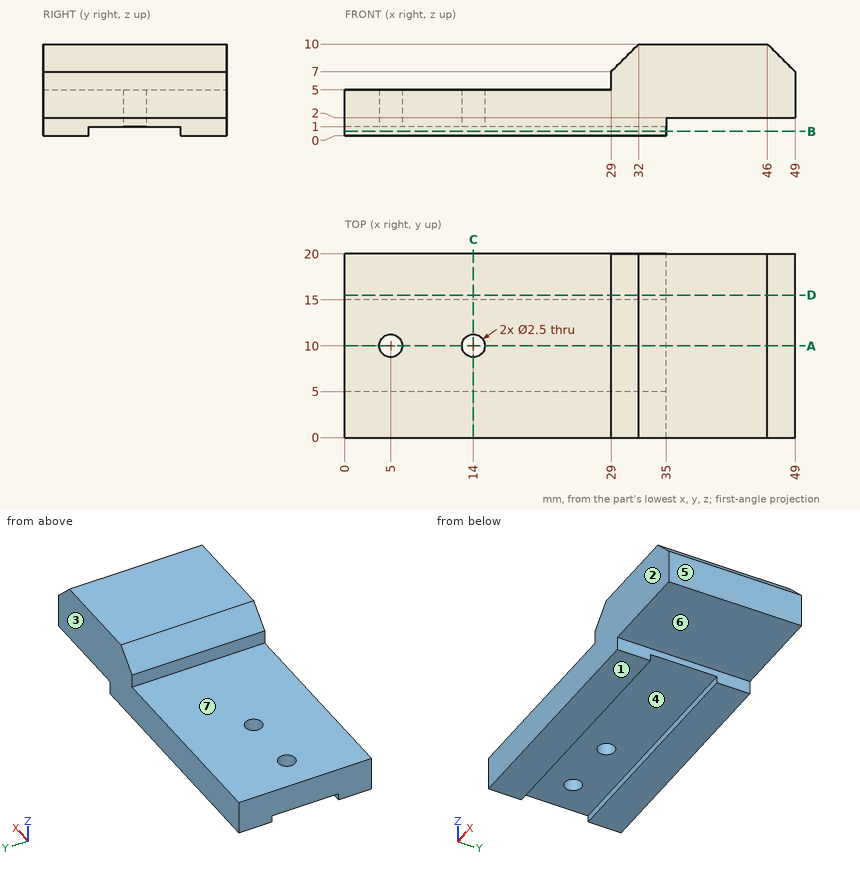
Part print with two shaded views. Sizes in mm from the minimum x, y, z corner. A direction names the side the tool comes from. Coordinates: 2 decimals unless noted, no trailing zeros. Order: outer loops, then holes, each group sorted by start corner. A loop starts at its lowest first (then second) coordinate and runs counter-clockwise, first axis right, second up.
(1) Saw through at D-D, the plane y = 15.5. Write the cut outline in (x, z).
Solution:
outline: (0, 0) - (35, 0) - (35, 2) - (49, 2) - (49, 7) - (46, 10) - (32, 10) - (29, 7) - (29, 5) - (0, 5) - close
(2) Saw through at C-C, the plane x = 14. Write the cut outline in (y, z).
Solution:
outline: (0, 0) - (5, 0) - (5, 1) - (8.75, 1) - (8.75, 5) - (0, 5) - close; (11.25, 1) - (15, 1) - (15, 0) - (20, 0) - (20, 5) - (11.25, 5) - close
(3) Pin check, flat tips, straight feed: pin 1 Ø0.6 at (y, z) = (5.5, 1) entering from +X; pin 2 Ø0.6 at (y, z) = (12, 6) entering from -X; pin 3 Ø5 at (x, y) = (21, 10) entering from +Z. Stop position of each tip, or through.
Solution:
pin 1: stops at x = 35
pin 2: stops at x = 29
pin 3: stops at z = 5
(4) Which spindle directions (+Z, -Z, +X, -X, +Y, -Y) get a long thin tool onto all of the face, cutting with end or side? Do the marked faces 5, 6 and 7. Say none if no direction does.
Solution:
face 5: +Z, -Z, +X, +Y, -Y
face 6: -Z, +X, +Y, -Y
face 7: +Z, -X, +Y, -Y
(5) Saw through at A-A, the plane y = 10. Write the cut outline in (x, z), and give its area (3 significant figures).
Solution:
outline: (0, 1) - (3.75, 1) - (3.75, 5) - (0, 5) - close; (6.25, 1) - (12.75, 1) - (12.75, 5) - (6.25, 5) - close; (15.25, 1) - (35, 1) - (35, 2) - (49, 2) - (49, 7) - (46, 10) - (32, 10) - (29, 7) - (29, 5) - (15.25, 5) - close
area: 253 mm2
(6) Saw through at B-B, the plane z = 0.5. Write the cut outline in (x, y).
Solution:
outline: (0, 0) - (35, 0) - (35, 5) - (0, 5) - close; (0, 15) - (35, 15) - (35, 20) - (0, 20) - close
(7) Drill centre lines: L1, parallel to Y at x = 14, z = 2.1; L2, parallel to Z at x = 43, y = 15.25; L3, parallel to Z at x = 13, y = 14.75. Where is each one in solid material? Low to high.
Solution:
L1: y = 0 to 8.75, 11.25 to 20
L2: z = 2 to 10
L3: z = 1 to 5
(8) Mould opens along Y. For the marked faces 1, 2, 3 and 4 say: released by +Y, released by -Y, zero draft, split by the parting line, or undercut.
Solution:
face 1: zero draft
face 2: released by -Y
face 3: released by +Y
face 4: undercut
